from build123d import *

# Parameters (mm, degrees)
EXTRUDE_1_DEPTH = 16
FILLET_1_R      = 10


with BuildPart() as part:
    # 草图1 → 凸台-拉伸1 (new body)
    with BuildSketch(Plane.XY):
        with BuildLine():
            Line((-132, 141.901665764), (-152, 141.901665764))
            Line((-152, 141.901665764), (-152, 194.51841477))
            Line((-152, 194.51841477), (-139.107955396, 203.545521584))
            Line((-139.107955396, 203.545521584), (-133.372191032, 195.354001142))
            ThreePointArc((-133.372191032, 195.354001142), (-116.5890905, 184.661986908), (-97.161250536, 188.969035335))
            Line((-97.161250536, 188.969035335), (84.690503297, 316.303004205))
            ThreePointArc((84.690503297, 316.303004205), (95.38251753, 333.086104737), (91.075469103, 352.513944702))
            Line((91.075469103, 352.513944702), (85.339704739, 360.705465145))
            Line((85.339704739, 360.705465145), (98.231749344, 369.732571959))
            Line((98.231749344, 369.732571959), (147.675320114, 351.736583923))
            Line((147.675320114, 351.736583923), (140.834917247, 332.942731507))
            Line((140.834917247, 332.942731507), (95.688258328, 208.903305564))
            Line((95.688258328, 208.903305564), (0, 141.901665764))
            Line((0, 141.901665764), (-132, 141.901665764))
        make_face()
    extrude(amount=EXTRUDE_1_DEPTH)

    # 圆角1
    fillet_1_edges = [part.edges().sort_by_distance(p)[0] for p in [
        (-152, 141.901665764, 8),
        (147.675320114, 351.736583923, 8),
        (95.688258328, 208.903305564, 8),
        (0, 141.901665764, 8),
    ]]
    fillet(fillet_1_edges, radius=FILLET_1_R)


solid = part.part
Work out the finished part from the listing and answer in its coordinate system (mm). A direction names the side the tool comes from. Round coordinates to 2 decimals unless told otherwise and drop trailing zeros. Write each loop counter-clockwise with the first axis right and the second up, starting at its lowest first coordinate (ties: lowest second). Pieces come first, ordered by that corner, then holes. Notation, with made-up numbers: (31, -5) -> (63, -5) arc R14 cw to (63, 14) -> close; hole circle Ø4 at (11, 47). An arc over 180 degrees is marked (long way). Answer as CSV lines item,"result". Start each with the question number.
(1) The part is cut by section A-A, the plane z = 3. Give the vertices of the cut face in (x, y), then the cut area to 3 significant figures.
(2) Each of these flat-tipped pins is pushed along its axis until it touches: pin 1 (2 mm diameter, centred on y = 223.5, z = 12.5, fed in from -X); pin 2 (2 mm diameter, centred on x = -69, z = 11.5, fed in from +Y); pin 3 (3 mm diameter, centred on x = 40.5, z = 8, fed in from +Y). Where does it stop, or does it pass through?
(3) Find the intervals of material crossed by probe 1 along X at (y, z) = (349, 9); probe 2 along Y at (x, z) = (91.5, 11.5); probe 3 along Y at (x, z) = (13.5, 10), in increasing order.
(4) The part is cut by section C-C, the plane y = 304.5. Give the vertices of the cut face in (x, z).
(5) The part is cut by section B-B, the plane x = -20.5. Give the vertices of the cut face in (y, z), then the cut area to 3 significant figures.
(6) A tool of negligible diameter and unlimited length cuts with its end or side. For faces 4 (the cylindrical face through (143.87, 350.09, 8.11)), 5 (the flat face through (88.25, 356.55, 7.89)), 6 (the flat face through (-136.28, 199.51, 7.89)), from which of +Z, -Z, +X, -X, +Y, -Y can it reach the whole face along a straight path? Write none if from no direction.
(7) The mould has two halves that part along Y. Classify faces 1 (the flat face through (48.48, 175.85, 7.89)), 2 (the cylindrical face through (95.33, 332.8, 7.89)), 3 (the flat face through (-152, 173, 8)): +Y half, -Y half, draft (parallel to the pull), parting line (faces both ways), or undercut.
Output values:
1,outline,"(-152, 151.9) arc R10 ccw to (-142, 141.9) -> (-3.15, 141.9) arc R10 ccw to (2.58, 143.71) -> (93.11, 207.09) arc R10 ccw to (96.77, 211.87) -> (144.26, 342.34) arc R10 ccw to (138.28, 355.16) -> (98.23, 369.73) -> (85.34, 360.71) -> (91.08, 352.51) arc R26 cw to (84.69, 316.3) -> (-97.16, 188.97) arc R26 cw to (-133.37, 195.35) -> (-139.11, 203.55) -> (-152, 194.52) -> close"
1,area,"25,900 mm²"
2,pin 1,"stops at x = -49.27"
2,pin 2,"stops at y = 209.39"
2,pin 3,"stops at y = 286.41"
3,probe 1,"x = 93.15 to 144.32"
3,probe 2,"y = 205.97 to 323.31, 351.89 to 365.02"
3,probe 3,"y = 151.35 to 266.45"
4,outline,"(67.83, 0) -> (130.48, 0) -> (130.48, 16) -> (67.83, 16) -> close"
5,outline,"(141.9, 0) -> (242.65, 0) -> (242.65, 16) -> (141.9, 16) -> close"
5,area,"1,610 mm²"
6,face 4,"+Z, -Z, +X"
6,face 5,"+Z, -Z, -X"
6,face 6,"+Z, -Z, +Y"
7,face 1,"-Y half"
7,face 2,"undercut"
7,face 3,"draft"
